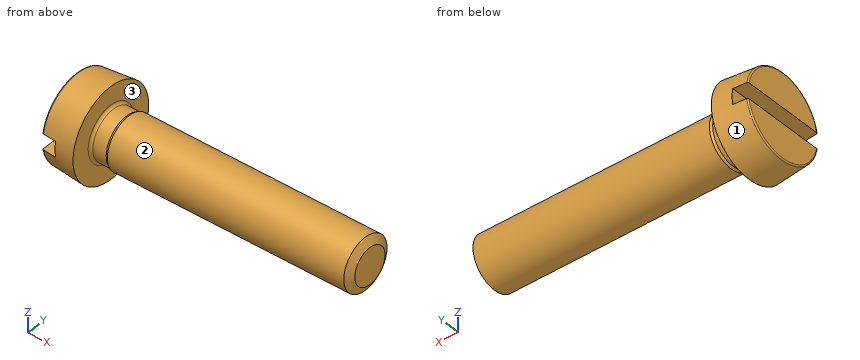
from build123d import *

# Parameters (mm, degrees)
CUT_EXTRUDE1_DEPTH = 1.1


with BuildPart() as part:
    # Sketch1 → Base-Revolve (revolve)
    with BuildSketch(Plane.XY, mode=Mode.PRIVATE) as base_revolve_sk:
        with BuildLine():
            Line((0, 0), (0, 3.180896357))
            ThreePointArc((0, 3.180896357), (0.026272266, 3.248455378), (0.091284426, 3.280515827))
            Line((0.091284426, 3.280515827), (2.6, 3.5))
            Line((2.6, 3.5), (2.6, 2.1))
            ThreePointArc((2.6, 2.1), (2.658578644, 1.958578644), (2.8, 1.9))
            Line((2.8, 1.9), (3.826794919, 1.9))
            Line((3.826794919, 1.9), (4, 2))
            Line((4, 2), (22.6, 2))
            Line((22.6, 2), (22.6, 0))
            Line((22.6, 0), (0, 0))
        make_face()
    revolve(base_revolve_sk.sketch.rotate(Axis((0, 0, 0), (1, 0, 0)), 90), axis=Axis((0, 0, 0), (1, 0, 0)))

    # Sketch2 → Cut-Extrude1 (cut)
    with BuildSketch(Plane.ZY):
        with BuildLine():
            Line((0.6, 3.44818793), (0.6, -3.44818793))
            ThreePointArc((0.6, -3.44818793), (0, -3.5), (-0.6, -3.44818793))
            Line((-0.6, -3.44818793), (-0.6, 3.44818793))
            ThreePointArc((-0.6, 3.44818793), (0, 3.5), (0.6, 3.44818793))
        make_face()
    extrude(amount=-CUT_EXTRUDE1_DEPTH, mode=Mode.SUBTRACT)

    # Sketch3 → Cut-Revolve1 (revolve, cut)
    with BuildSketch(Plane(origin=(0, 0, 0), x_dir=(1, 0, 0), z_dir=(0, 1, 0)), mode=Mode.PRIVATE) as cut_revolve1_sk:
        Polygon((22.250010267, 2), (22.949989733, 2), (22.6, 1.3938), align=None)
    revolve(cut_revolve1_sk.sketch.rotate(Axis((0, 0, 0), (1, 0, 0)), 180), axis=Axis((0, 0, 0), (1, 0, 0)), mode=Mode.SUBTRACT)


solid = part.part
Geometry check sheet. Reference: the model listing, model coordinates, mm. Face numbers are marked on the shaded views. Round coordinates to 2 decimals unless told otherwise and drop trailing zeros. Write each loop counter-clockwise with the first axis right and the second up, starting at its lowest first coordinate (ties: lowest second). Pieces come first, ordered by that corner, then holes. Notation, with made-up numbers: (86.5, 66.25) -> (131.5, 66.25) arc R35 ccw to (131.5, 104.25) -> close; hole circle Ø2 at (47.5, 21.25). An arc over 180 degrees is marked (long way). One line per item, written item: value. Start each with the question number.
(1) Go/stop test with flat-tipped pins: pin 1 Ø1.5 at (x, y) = (8.5, -0.5) entering from -Z; pin 2 Ø2 at (x, y) = (16.5, -2) entering from +Z; pin 3 Ø4 at (y, z) = (-0.5, 1) entering from -X; pin 4 Ø1 at (y, z) = (-1, 0) entering from -X. Record where each tip stops, or that it passes through.
(2) Draft check along X on the marked faces 1, 2 and 3. Enter one of: +X half, -X half, draft (parallel to the pull), parting line (faces both ways), or undercut.
(3) Cross-section at A-A, the plane y = 0. Record the cut outline in (x, z).
(4) Cross-section at C-C, the plane x = 8.25. Record the cut outline in (y, z), and give its area (3 significant figures).
(5) Scan lines: line 1 (X direction, y = -2.5, z = -0.25); line 2 (X direction, y = -2.5, z = -1); line 3 (Y direction, x = 16.75, z = 0). Record each from-to range of solid material in increasing order. Write a range as [from, to].
(6) Cross-section at B-B, the plane z = 0. Record the cut outline in (x, y), and give its area (3 significant figures).
Answer:
1. pin 1: z = -2
1. pin 2: z = 1.73
1. pin 3: x = 0
1. pin 4: x = 1.1
2. face 1: -X half
2. face 2: draft
2. face 3: +X half
3. outline: (0, -3.18) arc R0.1 ccw to (0.09, -3.28) -> (2.6, -3.5) -> (2.6, -2.1) arc R0.2 cw to (2.8, -1.9) -> (3.83, -1.9) -> (4, -2) -> (22.25, -2) -> (22.6, -1.39) -> (22.6, 1.39) -> (22.25, 2) -> (4, 2) -> (3.83, 1.9) -> (2.8, 1.9) arc R0.2 cw to (2.6, 2.1) -> (2.6, 3.5) -> (0.09, 3.28) arc R0.1 ccw to (0, 3.18) -> (0, 0.6) -> (1.1, 0.6) -> (1.1, -0.6) -> (0, -0.6) -> close
4. outline: circle Ø4 at (0, 0)
4. area: 12.6 mm²
5. line 1: [1.1, 2.6]
5. line 2: [0, 2.6]
5. line 3: [-2, 2]
6. outline: (1.1, -3.37) -> (2.6, -3.5) -> (2.6, -2.1) arc R0.2 cw to (2.8, -1.9) -> (3.83, -1.9) -> (4, -2) -> (22.25, -2) -> (22.6, -1.39) -> (22.6, 1.39) -> (22.25, 2) -> (4, 2) -> (3.83, 1.9) -> (2.8, 1.9) arc R0.2 cw to (2.6, 2.1) -> (2.6, 3.5) -> (1.1, 3.37) -> close
6. area: 89.8 mm²
